Part model, mm, in its own coordinate system. Face numbers are marked on the shaded views. A direction names the side the tool comes from. Coordinates: 2 decimals unless noted, no trailing zeros. Loops run counter-clockwise (first coordinate to the right, second up) from the corner with the lowest first, then second, coordinate; pieces in that order, holes last. Notation, with made-up numbers: (20, 53) -> (77, 53) arc R19 ccw to (77, 87) -> close; hole circle Ø9 at (22, 75.25). An arc over 180 degrees is marked (long way). One line per question, with ' | ' between items. Start each with the question number.
1) 3-axis set-ups, long thin cutter, end or side, ignore diameter. For the marked faces 5, 6 and 7: which of +Z, -Z, +X, -X, +Y, -Y reach the whole face in a straight line?
2) Cut at A-A (y = 0). List the corners of the cut face in (x, z), plus the area to 3 significant figures.
3) Cut at C-C (x = 8.75). List the corners of the cut face in (y, z).
4) Drop flat-ended pins along their axis: pin 1 (0.8 mm diameter, centred on x = -2.5, y = 0, fed in from -Z); pin 2 (1.6 mm diameter, centred on x = -3, y = 0, fed in from +Z); pin 3 (1.6 mm diameter, centred on x = -1.5, z = 0, fed in from +Y). Give the stop position or say it passes through.
5) Probe L1, parallel to X at y = -0.05, z = 0.6; L2, parallel to Y at x = -3, z = -0.7; L3, parallel to X at y = -1.15, z = 0.65. List the from-to ranges inside material, lowest first. Write a range as from..to.
6) Two-plate mould, pull along Z, no slides. Class the marked faces 1, 2, 3 and 4: released by +Z, released by -Z, zero draft, split by the parting line, or undercut.
7) Cut at B-B (z = 0). List the corners of the cut face in (x, y), plus the area to 3 significant figures.
8) Cut at D-D (x = 1.25). List the corners of the cut face in (y, z).
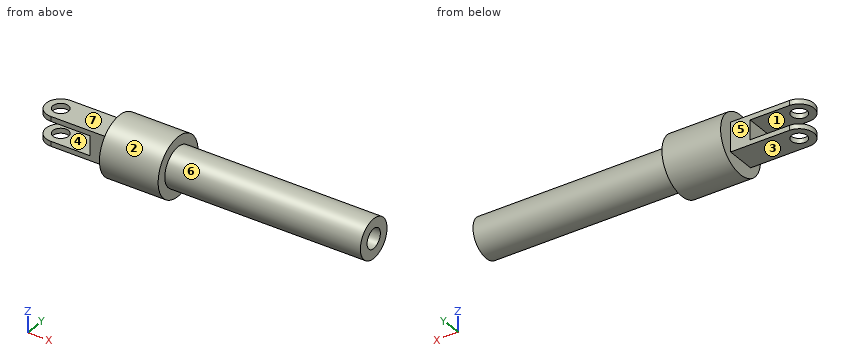
from build123d import *

# Parameters (mm, degrees)
SKETCH2_R           = 0.4
BOSS_EXTRUDE1_DEPTH = 0.75
CUT_EXTRUDE1_DEPTH  = 0.5
SKETCH4_R           = 0.5
CUT_EXTRUDE2_DEPTH  = 6


with BuildPart() as part:
    # Sketch1 → Revolve1 (revolve)
    with BuildSketch(Plane.XY, mode=Mode.PRIVATE) as revolve1_sk:
        Polygon((0, 0), (0, 1.5), (3, 1.5), (3, 1), (13, 1), (13, 0), align=None)
    revolve(revolve1_sk.sketch.rotate(Axis((0.124352332, 0, 0), (1, 0, 0)), 90), axis=Axis((0.124352332, 0, 0), (1, 0, 0)))

    # Sketch2 → Boss-Extrude1 (add, symmetric)
    with BuildSketch(Plane.XY):
        with BuildLine():
            Line((0, 0.75), (0, -0.75))
            Line((0, -0.75), (-3, -0.75))
            ThreePointArc((-3, -0.75), (-3.75, 0), (-3, 0.75))
            Line((-3, 0.75), (0, 0.75))
        make_face()
        with Locations((-3, 0)):
            Circle(SKETCH2_R, mode=Mode.SUBTRACT)
    extrude(amount=BOSS_EXTRUDE1_DEPTH, both=True)

    # Sketch3 → Cut-Extrude1 (cut, symmetric)
    with BuildSketch(Plane.XY):
        with BuildLine():
            Line((-1, 0.75), (-1, -0.75))
            Line((-1, -0.75), (-3, -0.75))
            ThreePointArc((-3, -0.75), (-3.75, 0), (-3, 0.75))
            Line((-3, 0.75), (-1, 0.75))
        make_face()
    extrude(amount=CUT_EXTRUDE1_DEPTH, both=True, mode=Mode.SUBTRACT)

    # Sketch4 → Cut-Extrude2 (cut)
    with BuildSketch(Plane(origin=(13, 0, 0), x_dir=(0, 0, -1), z_dir=(1, 0, 0))):
        Circle(SKETCH4_R)
    extrude(amount=-CUT_EXTRUDE2_DEPTH, mode=Mode.SUBTRACT)


solid = part.part
Reported:
1) face 5: +Z, -Z, -X, +Y | face 6: +X | face 7: +Z, -X, +Y, -Y
2) outline: (-3.75, -0.75) -> (-3.4, -0.75) -> (-3.4, -0.5) -> (-3.75, -0.5) -> close; (-3.75, 0.5) -> (-3.4, 0.5) -> (-3.4, 0.75) -> (-3.75, 0.75) -> close; (-2.6, -0.75) -> (0, -0.75) -> (0, -1.5) -> (3, -1.5) -> (3, -1) -> (13, -1) -> (13, -0.5) -> (7, -0.5) -> (7, 0.5) -> (13, 0.5) -> (13, 1) -> (3, 1) -> (3, 1.5) -> (0, 1.5) -> (0, 0.75) -> (-2.6, 0.75) -> (-2.6, 0.5) -> (-1, 0.5) -> (-1, -0.5) -> (-2.6, -0.5) -> close | area: 25.5 mm²
3) outline: circle Ø2 at (0, 0); hole circle Ø1 at (0, 0)
4) pin 1: stops at z = -0.75 | pin 2: stops at z = 0.75 | pin 3: stops at y = 0.75
5) L1: x = -3.75..-3.4, -2.6..13 | L2: y = -0.75..-0.4, 0.4..0.75 | L3: x = 0..3
6) face 1: undercut | face 2: split by the parting line | face 3: released by -Z | face 4: undercut
7) outline: (-1, -0.75) -> (0, -0.75) -> (0, -1.5) -> (3, -1.5) -> (3, -1) -> (13, -1) -> (13, -0.5) -> (7, -0.5) -> (7, 0.5) -> (13, 0.5) -> (13, 1) -> (3, 1) -> (3, 1.5) -> (0, 1.5) -> (0, 0.75) -> (-1, 0.75) -> close | area: 24.5 mm²
8) outline: circle Ø3 at (0, 0)
